from build123d import *

# Parameters (mm, degrees)
CHAMFER_1_SIZE = 1
CHAMFER_2_SIZE = 0.25


with BuildPart() as part:
    # 草图1 → 旋转1 (revolve)
    with BuildSketch(Plane.XY, mode=Mode.PRIVATE) as revolve_1_sk:
        Polygon((-4.124391585, 31), (5.875608415, 31), (5.875608415, 32.5), (8.875608415, 32.5), (8.875608415, 31), (184.875608415, 31), (184.875608415, 32.5), (187.875608415, 32.5), (187.875608415, 31), (197.875608415, 31), (197.875608415, 37.5), (-4.124391585, 37.5), align=None)
    revolve(revolve_1_sk.sketch.rotate(Axis((0, 0, 0), (1, 0, 0)), 90), axis=Axis((0, 0, 0), (1, 0, 0)))

    # 倒角1
    chamfer_1_edges = [part.edges().sort_by_distance(p)[0] for p in [
        (197.875608415, 0, -31),
        (197.875608415, 0, -37.5),
        (-4.124391585, 0, -37.5),
        (-4.124391585, 0, -31),
    ]]
    chamfer(chamfer_1_edges, length=CHAMFER_1_SIZE)

    # 倒角2
    chamfer_2_edges = [part.edges().sort_by_distance(p)[0] for p in [
        (8.875608415, 0, -31),
        (184.875608415, 0, -31),
    ]]
    chamfer(chamfer_2_edges, length=CHAMFER_2_SIZE)


solid = part.part
Model file for the job. Use its own axes, mm. A direction names the side the tool comes from. Give positions to 0.01 mm unless a question says otherwise; leave off trailing zeros. Write each loop counter-clockwise with the first axis right and the second up, starting at its lowest first coordinate (ties: lowest second). Pieces come first, ordered by that corner, then holes. Notation, with made-up numbers: M 15,-23.5 L 59,-23.5 A17 cw 59,-0.5 Z; hole C -35,87.25 d2. An arc over 180 degrees is marked long. One line per item, written item: value. Start each with the question number.
Q1. Probe probe 1 along Y at (x, z) = (108, 0); probe 2 along Z at (x, y) = (20, 1); probe 3 along Y at (x, z) = (8, 0). List the from-to ranges inside material, lowest first. Write a range as [from, to].
Q2. Two-plate mould, pull along X, no slides. Class faces 3 (the flat face through (5.876, 12, -29)), 4 (the cylindrical face through (98.104, -30.736, -4.036)), 5 (the flat face through (197.876, 32.3, 0.2)): +X half, -X half, draft (parallel to the pull), parting line (faces both ways), or undercut.
Q3. 3-axis set-ups, long thin cutter, end or side, ignore diameter. For faces 1 (the cylindrical face through (186.4, -9.76, 31)), 2 (the cylindrical face through (192.439, -30.736, -4.036)): which of +Z, -Z, +X, -X, +Y, -Y reach the whole face in a straight line?
Q4. Drop flat-ended pins along their axis: pin 1 Ø12 at (x, y) = (55.5, 28.5) entering from +Z; pin 2 Ø1.5 at (x, z) = (50, -25) entering from +Y; pin 3 Ø1 at (x, y) = (160, -28) entering from -Z; pin 4 Ø6 at (y, z) = (-18, 25.5) entering from +X. Give the stop position or say it passes through.
Q5. Saw through at A-A, the plane x = 44. Write the cut outline in (y, z), plus the area to 3 significant figures.
Output values:
1. probe 1: y = [-37.5, -31], [31, 37.5]
1. probe 2: z = [-37.49, -30.98], [30.98, 37.49]
1. probe 3: y = [-37.5, -32.5], [32.5, 37.5]
2. face 3: undercut
2. face 4: draft
2. face 5: +X half
3. face 1: none
3. face 2: +X, -X
4. pin 1: stops at z = 30
4. pin 2: stops at y = 28.6
4. pin 3: stops at z = -25.5
4. pin 4: stops at x = 197.88
5. outline: C 0,0 d75; hole C 0,0 d62
5. area: 1,400 mm²
